Could you check a few things on this model? Use its own coordinates, in mm. Face numbers are marked on the shaded views. A direction names the side the tool comes from. Give positions to 0.01 mm unless a question says otherwise; leave off trailing zeros. Loops run counter-clockwise (first coordinate to the right, second up) from the corner with the lowest first, then second, coordinate; pieces in that order, holes last. Notation, with made-up numbers: (-18.75, 7) -> (8.25, 7) arc R34 cw to (8.25, 43) -> close; hole circle Ø6 at (23, 8). An arc over 180 degrees is marked (long way). Put each result on its own line as item: value.
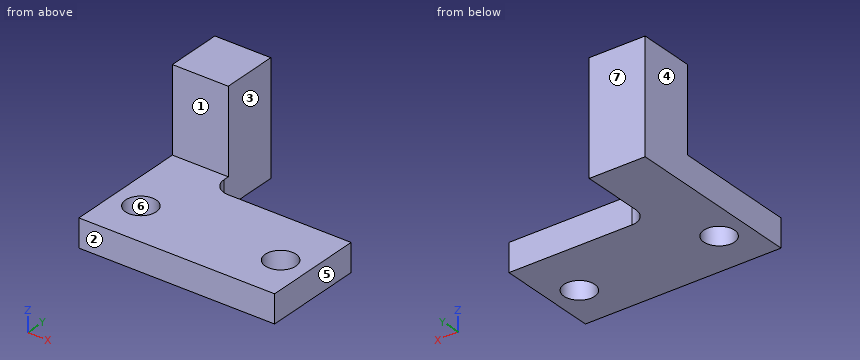
```python
from build123d import *

# Parameters (mm, degrees)
EXTRUDE_1_DEPTH     = 5
SKETCH_5_W          = 10
SKETCH_5_H          = 10
EXTRUDE_3_DEPTH     = 20
SKETCH_4_R          = 2.75
CUT_EXTRUDE_1_DEPTH = 20


with BuildPart() as part:
    # 草图1 → 凸台-拉伸1 (new body)
    with BuildSketch(Plane.XY):
        with BuildLine():
            Line((0, 0), (35, 0))
            Line((35, 0), (35, 18))
            Line((35, 18), (13, 18))
            ThreePointArc((13, 18), (10.878679656, 18.878679656), (10, 21))
            Line((10, 21), (10, 22))
            Line((10, 22), (0, 22))
            Line((0, 22), (0, 0))
        make_face()
    extrude(amount=EXTRUDE_1_DEPTH)

    # 草图5 → 凸台-拉伸3 (add)
    with BuildSketch(Plane(origin=(0, 0, 0), x_dir=(-1, 0, 0), z_dir=(0, 0, -1))):
        with Locations((-5, 27)):
            Rectangle(SKETCH_5_W, SKETCH_5_H)
    extrude(amount=-EXTRUDE_3_DEPTH)

    # 草图4 → 切除-拉伸1 (cut)
    with BuildSketch(Plane(origin=(0, 0, 0), x_dir=(-1, 0, 0), z_dir=(0, 0, -1))):
        with Locations((-30, 8)):
            Circle(SKETCH_4_R)
        with Locations((-5, 8)):
            Circle(SKETCH_4_R)
    extrude(amount=-CUT_EXTRUDE_1_DEPTH, mode=Mode.SUBTRACT)


solid = part.part
```
1. If we section it at C-C (y = 8): List the corners of the cut face in (x, z) for me.
Recorded:
outline: (0, 0) -> (2.25, 0) -> (2.25, 5) -> (0, 5) -> close; (7.75, 0) -> (27.25, 0) -> (27.25, 5) -> (7.75, 5) -> close; (32.75, 0) -> (35, 0) -> (35, 5) -> (32.75, 5) -> close
2. If we section it at B-B (z = 2.5): List the corners of the cut face in (x, y) for me, then the cut area to 3 significant figures.
Recorded:
outline: (0, 0) -> (35, 0) -> (35, 18) -> (13, 18) arc R3 cw to (10, 21) -> (10, 32) -> (0, 32) -> close; hole circle Ø5.5 at (5, 8); hole circle Ø5.5 at (30, 8)
area: 724 mm^2
3. If we section it at D-D (x = 30): List the corners of the cut face in (y, z) for me, then the cut area to 3 significant figures.
Recorded:
outline: (0, 0) -> (5.25, 0) -> (5.25, 5) -> (0, 5) -> close; (10.75, 0) -> (18, 0) -> (18, 5) -> (10.75, 5) -> close
area: 62.5 mm^2
4. I need wall thicknesses on line 1 (Y direction, x = 5, z = 3.6); line 2 (Y direction, x = 30, z = 1.2); line 3 (Z direction, x = 19, y = 2). Which ranges of each line are inside material? Lowest first, please.
Recorded:
line 1: y = 0 to 5.25, 10.75 to 32
line 2: y = 0 to 5.25, 10.75 to 18
line 3: z = 0 to 5
5. If we section it at A-A (x = 5): List the corners of the cut face in (y, z) for me, then the cut area to 4 significant figures.
Recorded:
outline: (0, 0) -> (5.25, 0) -> (5.25, 5) -> (0, 5) -> close; (10.75, 0) -> (32, 0) -> (32, 20) -> (22, 20) -> (22, 5) -> (10.75, 5) -> close
area: 282.5 mm^2
6. I'm going to push flat-ended pins straight in: pin 1 (6 mm diameter, centred on x = 11.5, z = 18, fed in from +Y); pin 2 (3 mm diameter, centred on y = 12, z = 7.5, fed in from -X); pin 3 (1.5 mm diameter, centred on x = 7, z = 8, fed in from -Y); pin 4 (3.5 mm diameter, centred on y = 27, z = 7, fed in from +X). Where does each tip first touch, or does it pass through?
Recorded:
pin 1: stops at y = 32
pin 2: passes through
pin 3: stops at y = 22
pin 4: stops at x = 10
7. For the marked faces 1, 2 and 3, which set-ups out of +Z, -Z, +X, -X, +Y, -Y let a thin tool reach every point of the face, with its end or its side?
Recorded:
face 1: +Z, +X, -X, -Y
face 2: +Z, -Z, +X, -X, -Y
face 3: +Z, -Z, +X, +Y
8. Thinking about a two-plate mould opening in X: for the marked faces 4, 5, 6 and 7, which applies, pulls with the +X half, pulls with the -X half, needs draft (parallel to the pull), parting line crosses it, or undercut?
Recorded:
face 4: pulls with the -X half
face 5: pulls with the +X half
face 6: undercut
face 7: needs draft
